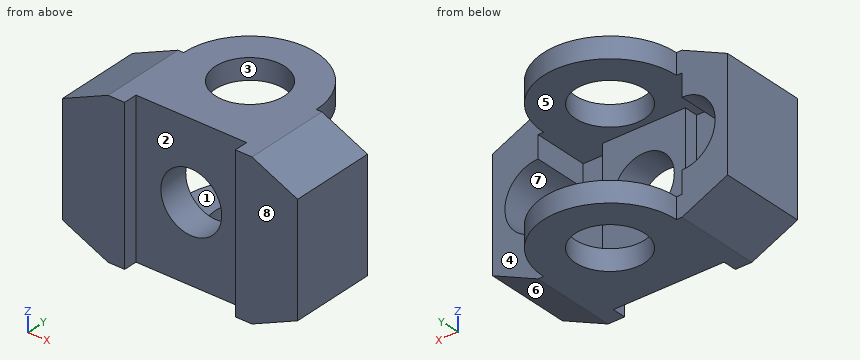
```python
from build123d import *

# Parameters (mm, degrees)
BASE_BLOCK_DEPTH           = 31
LUG_A_DEPTH                = 7.5
LUG_START                  = -7.5
LUG_A_WEB_DEPTH            = 7.5
BORE_25_PROFILE_R          = 12.5
BORE_25_DEPTH              = 89.635489506
LUG_B_BASE_DEPTH           = 11
LUG_B_PROFILE_W            = 30
LUG_B_PROFILE_H            = 40
LUG_B_DEPTH                = 5
BORE_22_REACH              = 65.902
BORE_22_PROFILE_R          = 11
RELIEF_SLOT_40X5_REACH     = 90.635
RELIEF_SLOT_40X5_PROFILE_W = 40
RELIEF_SLOT_40X5_PROFILE_H = 5


with BuildPart() as part:
    # Base Block Profile → Base Block (new body)
    with BuildSketch(Plane(origin=(0, 0, 0), x_dir=(1, 0, 0), z_dir=(0, 1, 0))):
        Polygon((-26, 27.5), (26, 27.5), (42.5, 20), (42.5, -20), (26, -27.5), (-26, -27.5), (-42.5, -20), (-42.5, 20), align=None)
        with BuildLine():
            Line((-26, 20), (26, 20))
            Line((26, 20), (26, 12))
            ThreePointArc((26, 12), (38, 0), (26, -12))
            Line((26, -12), (26, -20))
            Line((26, -20), (-26, -20))
            Line((-26, -20), (-26, -12))
            ThreePointArc((-26, -12), (-38, 0), (-26, 12))
            Line((-26, 12), (-26, 20))
        make_face(mode=Mode.SUBTRACT)
    extrude(amount=BASE_BLOCK_DEPTH)

    # Lug A Profile → Lug A (add)
    with BuildSketch(Plane.XY.offset(27.5)):
        with BuildLine():
            Line((-24, 31), (24, 31))
            ThreePointArc((24, 31), (0, 55), (-24, 31))
        make_face()
    extrude(amount=-LUG_A_DEPTH)

    # Lug A Web Profile → Lug A Web (add)
    with BuildSketch(Plane(origin=(0, 0, -27.5), x_dir=(-1, 0, 0), z_dir=(0, 0, -1)).offset(LUG_START)):
        with BuildLine():
            Line((-24, 31), (24, 31))
            ThreePointArc((24, 31), (0, 55), (-24, 31))
        make_face()
    extrude(amount=LUG_A_WEB_DEPTH)

    # Bore _25 Profile → Bore _25 (cut, through all)
    with BuildSketch(Plane.XY.offset(27.5)):
        with Locations((0, 31)):
            Circle(BORE_25_PROFILE_R)
    extrude(amount=-BORE_25_DEPTH, mode=Mode.SUBTRACT)

    # Lug B Base Profile → Lug B Base (add)
    with BuildSketch(Plane(origin=(0, 0, 0), x_dir=(1, 0, 0), z_dir=(0, 1, 0))):
        Polygon((42.5, 20), (26, 27.5), (-26, 27.5), (-42.5, 20), (-42.5, -20), (-26, -27.5), (26, -27.5), (42.5, -20), align=None)
    extrude(amount=LUG_B_BASE_DEPTH)

    # Lug B Profile → Lug B (add)
    with BuildSketch(Plane(origin=(0, 11, 0), x_dir=(1, 0, 0), z_dir=(0, 1, 0))):
        Rectangle(LUG_B_PROFILE_W, LUG_B_PROFILE_H)
    extrude(amount=LUG_B_DEPTH)

    # Bore _22 Profile → Bore _22 (cut, up to next)
    with BuildSketch(Plane(origin=(0, 16, 0), x_dir=(1, 0, 0), z_dir=(0, 1, 0)), mode=Mode.PRIVATE) as bore_22_sk1:
        with Locations(Location((0, 0, 0), (0, 0, 270))):
            Circle(BORE_22_PROFILE_R)
    bore_22_tool1 = extrude(bore_22_sk1.sketch, amount=-BORE_22_REACH, mode=Mode.PRIVATE) & part.part
    add(bore_22_tool1.solids().sort_by_distance((0, 16, 0))[0], mode=Mode.SUBTRACT)

    # Relief Slot 40x5 Profile → Relief Slot 40x5 (cut, up to next)
    with BuildSketch(Plane.XY.offset(27.5), mode=Mode.PRIVATE) as relief_slot_40x5_sk1:
        with Locations((0, 2.5)):
            Rectangle(RELIEF_SLOT_40X5_PROFILE_W, RELIEF_SLOT_40X5_PROFILE_H)
    relief_slot_40x5_tool1 = extrude(relief_slot_40x5_sk1.sketch, amount=-RELIEF_SLOT_40X5_REACH, mode=Mode.PRIVATE) & part.part
    add(relief_slot_40x5_tool1.solids().sort_by_distance((0, 2.5, 27.5))[0], mode=Mode.SUBTRACT)


solid = part.part
```
Work out the finished part from the listing and answer in its coordinate system (mm). Face numbers are marked on the shaded views. A direction names the side the tool comes from. Coordinates: 2 decimals unless noted, no trailing zeros. Loops run counter-clockwise (first coordinate to the right, second up) from the corner with the lowest first, then second, coordinate; pieces in that order, holes last.
1) Section C-C (y = 7) is taken. Give the vertices of the cut face in (x, z).
Results:
outline: (-42.5, -20) - (-26, -27.5) - (26, -27.5) - (42.5, -20) - (42.5, 20) - (26, 27.5) - (-26, 27.5) - (-42.5, 20) - close; hole circle Ø22 at (0, 0)
2) Section B-B (x = 0) is taken. Give the vertices of the cut face in (y, z).
Results:
outline: (5, -27.5) - (18.5, -27.5) - (18.5, -20) - (16, -20) - (16, -11) - (5, -11) - close; (5, 11) - (16, 11) - (16, 20) - (18.5, 20) - (18.5, 27.5) - (5, 27.5) - close; (43.5, -27.5) - (55, -27.5) - (55, -20) - (43.5, -20) - close; (43.5, 20) - (55, 20) - (55, 27.5) - (43.5, 27.5) - close
3) Section D-D (z = 0) is taken. Give the vertices of the cut face in (x, y).
Results:
outline: (-42.5, 0) - (-20, 0) - (-20, 5) - (-11, 5) - (-11, 16) - (-15, 16) - (-15, 11) - (-38, 11) - (-38, 31) - (-42.5, 31) - close; (11, 5) - (20, 5) - (20, 0) - (42.5, 0) - (42.5, 31) - (38, 31) - (38, 11) - (15, 11) - (15, 16) - (11, 16) - close
4) Section A-A (z = -22.5) is taken. Give the vertices of the cut face in (x, y), plus the area to 3 significant figures.
Results:
outline: (-37, 0) - (-20, 0) - (-20, 5) - (20, 5) - (20, 0) - (37, 0) - (37, 31) - (24, 31) arc R24 ccw to (-24, 31) - (-37, 31) - close; hole circle Ø25 at (0, 31)
area: 2,510 mm2
5) Flat-ended cylindrical pins translate along their axes: pin 1 (22 mm diameter, centred on x = 3, y = 35.5, fed in from -Z); pin 2 (11.5 mm diameter, centred on x = 29.5, z = -4.5, fed in from +Y); pin 3 (5 mm diameter, centred on x = 5.5, z = 7, fed in from -Y); pin 4 (15 mm diameter, centred on x = -0.5, z = -7, fed in from +Y). Find the tip coordinate at first contact, or state that the pin passes through.
Results:
pin 1: stops at z = -27.5
pin 2: stops at y = 11
pin 3: stops at y = 5
pin 4: stops at y = 16
6) For the marked faces 1, 2, 3 and 4, determine the directions among +Z, -Z, +X, -X, +Y, -Y from which every point of the face is accessible in a straight line to the end or side of a thin tool.
Results:
face 1: +Y
face 2: +Z, -Z, -Y
face 3: +Z, -Z
face 4: +Z, -Z, +X, +Y
7) For a pull along Z with two mould halves and no side action, classify the marked faces 5, 6, 7 and 8 as +Z half, -Z half, draft (parallel to the pull), parting line (faces both ways), or undercut.
Results:
face 5: undercut
face 6: -Z half
face 7: undercut
face 8: draft
8) Consider probe 1 along X at (y, z) = (12.25, 0); probe 2 along Y at (x, z) = (0, -25.5); probe 3 along X at (y, z) = (31.5, -25). Determine where each line is inside the solid, lowest interval first.
Results:
probe 1: x = -42.5 to -38, -15 to -11, 11 to 15, 38 to 42.5
probe 2: y = 5 to 18.5, 43.5 to 55
probe 3: x = -23.99 to -12.49, 12.49 to 23.99
